Geometry: final body of the model. Coordinates: model frame, mm. A direction names the side the tool comes from. Give positions to 0.01 mm unless a question says otherwise; leave off trailing zeros. Loops run counter-clockwise (first coordinate to the right, second up) from the corner with the lowest first, then second, coordinate; pieces in that order, holes last. Notation, with made-up numbers: (0, 30) -> (10, 30) arc R5 ccw to (10, 39) -> close; hole circle Ø11 at (-29, 82). An arc over 180 degrees is marked (long way). Answer in a Markdown table with one row per item. Add a question column.
1) Section query A-A (x = 10). Return the cut outline in (y, z), plus the area to 3 significant figures.
2) Section query C-C (z = 3.5). Return the cut outline in (x, y), plus the area to 3 significant figures.
3) Section query D-D (z = 6.5). Return the cut outline in (x, y), plus the area to 3 significant figures.
4) Draft query along Y for faces 3 (the cylindrical face through (67.395, -22.073, 5.108)), 4 (the flat face through (37, 0, 1)), 5 (the flat face through (75, -21, 3)), 6 (the flat face through (67.395, -22.479, 0.126)). Return one class per face: +Y half, -Y half, draft (parallel to the pull), parting line (faces both ways), or undercut.
5) Line query: line 1 (X direction, y = -20.75, z = 5.25); line 2 (Y direction, x = 11, z = 4.75); line 3 (Z direction, x = 3, y = -24.75). Output: solid intervals per line, ascending. Write a range as from..to.
6) First-contact query: P1, Ø1.6, axis at x = 23.5, z = 1, coming from the -Y side; P2, Ø4, axis at x = 37.5, y = -10, coming from the -Z side; P3, Ø1.5, axis at x = 25.5, y = -18.5, coming from the +Z side; P4, Ø1.5, axis at x = 43, y = -21, coming from the -Z side. Flat tips, straight axial feed; report the tip coordinate or a pass-through.
7) Access query for faces 1 (the flat face through (0, -18.9, 1.5)), 2 (the flat face through (45, -22.5, 2.5)). Directions: +Z, -Z, +X, -X, +Y, -Y. A direction counts if a zero-diameter tool reaches every point of the face in a straight line with its end or side. Return the directions, or none.
8) Section query B-B (y = -10). Return the cut outline in (x, z).
```python
from build123d import *

# Parameters (mm, degrees)
SKETCH1_W           = 75
SKETCH1_H           = 20
SKETCH1_R           = 2.5
BOSS_EXTRUDE1_DEPTH = 2
BOSS_EXTRUDE2_DEPTH = 15
LPATTERN1_COUNT     = 3
LPATTERN1_PITCH     = 30
FILLET1_R           = 5


with BuildPart() as part:
    # Sketch1 → Boss-Extrude1 (new body)
    with BuildSketch(Plane.XY):
        with Locations((37.5, -10)):
            Rectangle(SKETCH1_W, SKETCH1_H)
        with Locations((10, -10)):
            Circle(SKETCH1_R, mode=Mode.SUBTRACT)
        with Locations((65, -10)):
            Circle(SKETCH1_R, mode=Mode.SUBTRACT)
        with Locations((37.5, -10)):
            Circle(SKETCH1_R, mode=Mode.SUBTRACT)
    extrude(amount=BOSS_EXTRUDE1_DEPTH)

    # Sketch2 → Boss-Extrude2 (add)
    # profile 1 of 2: a face of its own
    with BuildSketch(Plane.ZY):
        with BuildLine():
            ThreePointArc((2, -28.361951712), (9.25, -24.8), (2, -21.238048288))
            Line((2, -21.238048288), (2, -24.8))
            Line((2, -24.8), (2, -28.361951712))
        make_face()
        with BuildLine():
            ThreePointArc((7.5, -24.8), (4.75, -27.55), (2, -24.8))
            ThreePointArc((2, -24.8), (4.75, -22.05), (7.5, -24.8))
        make_face(mode=Mode.SUBTRACT)
    # profile 2 of 2: a face of its own
    with BuildSketch(Plane.ZY):
        with BuildLine():
            Line((2, -21.238048288), (2, -20))
            Line((2, -20), (0, -20))
            Line((0, -20), (0.255811418, -25.028624118))
            ThreePointArc((0.255811418, -25.028624118), (0.762853744, -26.886304085), (2, -28.361951712))
            Line((2, -28.361951712), (2, -24.8))
            Line((2, -24.8), (2, -21.238048288))
        make_face()
    boss_extrude2 = extrude(amount=-BOSS_EXTRUDE2_DEPTH)

    # LPattern1: Boss-Extrude2 ×3
    with Locations(*[(i * LPATTERN1_PITCH, 0, 0) for i in range(1, LPATTERN1_COUNT)]):
        add(boss_extrude2)

    # Fillet1
    fillet1_edges = [part.edges().sort_by_distance(p)[0] for p in [
        (0, 0, 1),
        (75, 0, 1),
    ]]
    fillet(fillet1_edges, radius=FILLET1_R)


solid = part.part
```
Evaluation:
| question | item | result |
|---|---|---|
| 1 | outline | (-25.03, 0.26) -> (-20, 0) -> (-12.5, 0) -> (-12.5, 2) -> (-21.24, 2) arc R4.5 ccw (long way) to start; (-7.5, 0) -> (0, 0) -> (0, 2) -> (-7.5, 2) -> close; hole circle Ø5.5 at (-24.8, 4.75) |
| 1 | area | 74.5 mm² |
| 2 | outline | (0, -29.12) -> (15, -29.12) -> (15, -27.25) -> (0, -27.25) -> close; (0, -22.35) -> (15, -22.35) -> (15, -20.48) -> (0, -20.48) -> close; (30, -29.12) -> (45, -29.12) -> (45, -27.25) -> (30, -27.25) -> close; (30, -22.35) -> (45, -22.35) -> (45, -20.48) -> (30, -20.48) -> close; (60, -29.12) -> (75, -29.12) -> (75, -27.25) -> (60, -27.25) -> close; (60, -22.35) -> (75, -22.35) -> (75, -20.48) -> (60, -20.48) -> close |
| 2 | area | 169 mm² |
| 3 | outline | (0, -28.95) -> (15, -28.95) -> (15, -26.92) -> (0, -26.92) -> close; (0, -22.68) -> (15, -22.68) -> (15, -20.65) -> (0, -20.65) -> close; (30, -28.95) -> (45, -28.95) -> (45, -26.92) -> (30, -26.92) -> close; (30, -22.68) -> (45, -22.68) -> (45, -20.65) -> (30, -20.65) -> close; (60, -28.95) -> (75, -28.95) -> (75, -26.92) -> (60, -26.92) -> close; (60, -22.68) -> (75, -22.68) -> (75, -20.65) -> (60, -20.65) -> close |
| 3 | area | 182 mm² |
| 4 | face 3 | undercut |
| 4 | face 4 | +Y half |
| 4 | face 5 | draft |
| 4 | face 6 | -Y half |
| 5 | line 1 | 0..15, 30..45, 60..75 |
| 5 | line 2 | -29.3..-27.55, -22.05..-20.3 |
| 5 | line 3 | 0.24..2, 7.5..9.25 |
| 6 | P1 | y = -20 |
| 6 | P2 | through |
| 6 | P3 | z = 2 |
| 6 | P4 | z = 0.01 |
| 7 | face 1 | +Z, -Z, -X, +Y, -Y |
| 7 | face 2 | +Z, -Z, -Y |
| 8 | outline | (0, 0) -> (7.5, 0) -> (7.5, 2) -> (0, 2) -> close; (12.5, 0) -> (35, 0) -> (35, 2) -> (12.5, 2) -> close; (40, 0) -> (62.5, 0) -> (62.5, 2) -> (40, 2) -> close; (67.5, 0) -> (75, 0) -> (75, 2) -> (67.5, 2) -> close |
